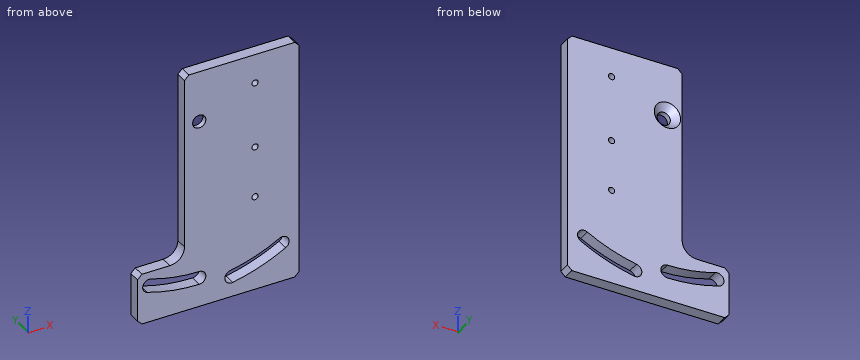
```python
from build123d import *

# Parameters (mm, degrees)
SKETCH_1_W                   = 110
SKETCH_1_H                   = 165
EXTRUDE_1_DEPTH              = 8
SKETCH_2_W                   = 32
SKETCH_2_H                   = 130
CUT_EXTRUDE_1_DEPTH          = 8
HOLE_WIZARD_M8_1_D           = 9
HOLE_WIZARD_M8_1_DEPTH       = 10
HOLE_WIZARD_M8_1_CSINK_D     = 17.92
HOLE_WIZARD_M8_1_CSINK_ANGLE = 90
HOLE_WIZARD_M8_1_TIP         = 2.703872786
CUT_EXTRUDE_2_DEPTH          = 8
CUT_EXTRUDE_3_DEPTH          = 8
CHAMFER_1_SIZE               = 3
HOLE_WIZARD_M5_1_D           = 4.2
FILLET_1_R                   = 10


with BuildPart() as part:
    # 草图1 → 凸台-拉伸1 (new body)
    with BuildSketch(Plane(origin=(0, 0, 0), x_dir=(1, 0, 0), z_dir=(0, 1, 0))):
        Rectangle(SKETCH_1_W, SKETCH_1_H)
    extrude(amount=EXTRUDE_1_DEPTH)

    # 草图2 → 切除-拉伸1 (cut)
    with BuildSketch(Plane(origin=(0, 8, 0), x_dir=(1, 0, 0), z_dir=(0, 1, 0))):
        with Locations((-39, -17.5)):
            Rectangle(SKETCH_2_W, SKETCH_2_H)
    extrude(amount=-CUT_EXTRUDE_1_DEPTH, mode=Mode.SUBTRACT)

    # M8 六角凹锥坑螺钉的锥形沉头孔1
    with Locations(Plane(origin=(0, 8, 0), x_dir=(1, 0, 0), z_dir=(0, 1, 0))):
        with Locations((-13, -47.5)):
            CounterSinkHole(HOLE_WIZARD_M8_1_D / 2, HOLE_WIZARD_M8_1_CSINK_D / 2, depth=HOLE_WIZARD_M8_1_DEPTH, counter_sink_angle=HOLE_WIZARD_M8_1_CSINK_ANGLE)
            with Locations((0, 0, -(HOLE_WIZARD_M8_1_DEPTH + HOLE_WIZARD_M8_1_TIP / 2))):  # 118° drill point
                Cone(0, HOLE_WIZARD_M8_1_D / 2, HOLE_WIZARD_M8_1_TIP, mode=Mode.SUBTRACT)

    # 草图6 → 切除-拉伸2 (cut)
    with BuildSketch(Plane(origin=(0, 8, 0), x_dir=(1, 0, 0), z_dir=(0, 1, 0))):
        with BuildLine():
            ThreePointArc((-13, 67), (-30.911746247, 65.590314998), (-48.382445856, 61.395971116))
            ThreePointArc((-48.382445856, 61.395971116), (-51.271623705, 55.725640318), (-45.601292907, 52.836462469))
            ThreePointArc((-45.601292907, 52.836462469), (-29.503836062, 56.701119933), (-13, 58))
            ThreePointArc((-13, 58), (-8.5, 62.5), (-13, 67))
        make_face()
    extrude(amount=-CUT_EXTRUDE_2_DEPTH, mode=Mode.SUBTRACT)

    # 草图6<3> → 切除-拉伸3 (cut)
    with BuildSketch(Plane(origin=(0, 8, 0), x_dir=(1, 0, 0), z_dir=(0, 1, 0))):
        with BuildLine():
            ThreePointArc((-13, 67), (-30.911746247, 65.590314998), (-48.382445856, 61.395971116))
            ThreePointArc((-48.382445856, 61.395971116), (-51.271623705, 55.725640318), (-45.601292907, 52.836462469))
            ThreePointArc((-45.601292907, 52.836462469), (-29.503836062, 56.701119933), (-13, 58))
            ThreePointArc((-13, 58), (-8.5, 62.5), (-13, 67))
        make_face()
        with BuildLine():
            ThreePointArc((45.83353556, 59.947033898), (28.30077784, 67.827775275), (9.751057901, 72.868764073))
            ThreePointArc((9.751057901, 72.868764073), (4.493595053, 69.282807519), (8.079551606, 64.025344671))
            ThreePointArc((8.079551606, 64.025344671), (25.266434979, 59.354714234), (41.511071723, 52.052966102))
            ThreePointArc((41.511071723, 52.052966102), (47.61933754, 53.838768081), (45.83353556, 59.947033898))
        make_face()
    extrude(amount=-CUT_EXTRUDE_3_DEPTH, mode=Mode.SUBTRACT)

    # 倒角1
    chamfer_1_edges = [part.edges().sort_by_distance(p)[0] for p in [
        (-55, 4, -47.5),
        (-23, 4, 82.5),
        (55, 4, 82.5),
        (-55, 4, -82.5),
        (55, 4, -82.5),
    ]]
    chamfer(chamfer_1_edges, length=CHAMFER_1_SIZE)

    # M5 螺纹孔1 (through all)
    with Locations(Plane(origin=(0, 8, 0), x_dir=(1, 0, 0), z_dir=(0, 1, 0))):
        with Locations((25, -62.5), (25, -17.5), (25, 17.5)):
            Hole(HOLE_WIZARD_M5_1_D / 2)

    # 圆角1
    fillet_1_edges = [part.edges().sort_by_distance(p)[0] for p in [
        (-23, 4, -47.5),
    ]]
    fillet(fillet_1_edges, radius=FILLET_1_R)


solid = part.part
```
The listing builds one solid part. Answer for the finished solid, in the listing's coordinates (mm). Give positions to 0.01 mm unless a question says otherwise; leave off trailing zeros. Order: outer loops, then holes, each group sorted by start corner. A loop starts at its lowest first (then second) coordinate and runs counter-clockwise, first axis right, second up. Notation, with made-up numbers: (70, 10.25) - (128, 10.25) arc R34 ccw to (128, 40.25) - close; hole circle Ø4 at (63, -0.5). An arc over 180 degrees is marked (long way). Answer in a Markdown table with one row per item. Add a question column.
Q1. Given P1, Ø4, axis at y = 6, z = -3.5, coming from the -X side; P2, Ø5.5, axis at x = 25, z = 17.5, coming from the +Y side; P3, Ø4, axis at x = -42.5, y = 4, coming from the +Z side, each flat-ended and moving along its own axis, determine where each tip first touches the part or whether it passes through.
Q2. The part is cut by section C-C (z = -56). Determine the outline of the cut face in (x, y), then the cut area to 3 significant figures.
Q3. Find the intervals of material crossed by line 1 along X through (y, z) = (2.5, 62.5); line 2 along X through (y, z) = (2.35, 47.5); line 3 along Z through (x, y) = (25, 5.5), in increasing order. Write a range as [from, to].
Q4. The part is cut by section B-B (z = 62.5). Determine the outline of the cut face in (x, y), then the cut area to 3 significant figures.
Q5. The part is cut by section D-D (x = 12). Determine the outline of the cut face in (y, z), then the cut area to 3 significant figures.
Q6. The part is cut by section A-A (y = 5.5). Determine the outline of the cut face in (x, z), then the cut area to 3 significant figures.
Determined:
| question | item | result |
|---|---|---|
| 1 | P1 | stops at x = -23 |
| 1 | P2 | stops at y = 8 |
| 1 | P3 | stops at z = -47.5 |
| 2 | outline | (-55, 0) - (-51.35, 0) - (-51.35, 8) - (-55, 8) - close; (-33.45, 0) - (33.58, 0) - (33.58, 8) - (-33.45, 8) - close; (48.17, 0) - (55, 0) - (55, 8) - (48.17, 8) - close |
| 2 | area | 620 mm² |
| 3 | line 1 | x = [-23, 22.9], [27.1, 55] |
| 3 | line 2 | x = [-23, -17.5], [-8.5, 55] |
| 3 | line 3 | z = [-82.5, -68.96], [-59.45, -19.6], [-15.4, 15.4], [19.6, 60.4], [64.6, 82.5] |
| 4 | outline | (-23, 0) - (22.9, 0) - (22.9, 8) - (-23, 8) - close; (27.1, 0) - (55, 0) - (55, 8) - (27.1, 8) - close |
| 4 | area | 590 mm² |
| 5 | outline | (0, -82.5) - (8, -82.5) - (8, -72.42) - (0, -72.42) - close; (0, -63.21) - (8, -63.21) - (8, 82.5) - (0, 82.5) - close |
| 5 | area | 1,250 mm² |
| 6 | outline | (-55, -79.5) - (-52, -82.5) - (52, -82.5) - (55, -79.5) - (55, 79.5) - (52, 82.5) - (-20, 82.5) - (-23, 79.5) - (-23, -37.5) arc R10 cw to (-33, -47.5) - (-52, -47.5) - (-55, -50.5) - close; hole (-48.38, -61.4) arc R114.5 ccw to (-13, -67) arc R4.5 ccw to (-13, -58) arc R105.5 cw to (-45.6, -52.84) arc R4.5 ccw to start; hole circle Ø12.92 at (-13, 47.5); hole (8.08, -64.03) arc R4.5 ccw to (9.75, -72.87) arc R122.5 ccw to (45.83, -59.95) arc R4.5 ccw to (41.51, -52.05) arc R113.5 cw to start; hole circle Ø4.2 at (25, -17.5); hole circle Ø4.2 at (25, 17.5); hole circle Ø4.2 at (25, 62.5) |
| 6 | area | 13,000 mm² |
